The listing builds one solid part. Answer for the finished solid, in the listing's coordinates (mm). A direction names the side the tool comes from. Coordinates: 2 decimals unless noted, no trailing zeros. Order: outer loops, then holes, each group sorted by start corner. A loop starts at its lowest first (then second) coordinate and runs counter-clockwise, first axis right, second up. Notation, with made-up numbers: (23, 21.25) -> (73, 21.25) arc R28 cw to (73, 56.25) -> close; hole circle Ø2 at (-27, 36). An arc over 180 degrees is marked (long way). Write item = value, one per line. Start each with the question number.
```python
from build123d import *

# Parameters (mm, degrees)
SKETCH_1_R      = 32.5
EXTRUDE_1_DEPTH = 25
SKETCH_2_R      = 34.5
SKETCH_2_R_2    = 32.5
EXTRUDE_2_DEPTH = 20
FILLET_1_R      = 1
CHAMFER_1_SIZE  = 2


with BuildPart() as part:
    # 草图1 → 凸台-拉伸1 (new, symmetric)
    with BuildSketch(Plane(origin=(0, 0, 0), x_dir=(0, 0, -1), z_dir=(1, 0, 0))):
        Circle(SKETCH_1_R)
        with BuildLine():
            Line((5, 17.291616466), (5, 20.591616466))
            Line((5, 20.591616466), (-5, 20.591616466))
            Line((-5, 20.591616466), (-5, 17.291616466))
            ThreePointArc((-5, 17.291616466), (0, -18), (5, 17.291616466))
        make_face(mode=Mode.SUBTRACT)
    extrude(amount=EXTRUDE_1_DEPTH, both=True)

    # 草图2 → 凸台-拉伸2 (add, symmetric)
    with BuildSketch(Plane(origin=(0, 0, 0), x_dir=(0, 0, -1), z_dir=(1, 0, 0))):
        Circle(SKETCH_2_R)
        Circle(SKETCH_2_R_2, mode=Mode.SUBTRACT)
    extrude(amount=EXTRUDE_2_DEPTH, both=True)

    # 圆角1
    fillet_1_edges = [part.edges().sort_by_distance(p)[0] for p in [
        (-20, 0, 32.5),
        (20, 0, 32.5),
    ]]
    fillet(fillet_1_edges, radius=FILLET_1_R)

    # 倒角1
    chamfer_1_edges = [part.edges().sort_by_distance(p)[0] for p in [
        (-25, 0, 32.5),
        (25, 0, 32.5),
    ]]
    chamfer(chamfer_1_edges, length=CHAMFER_1_SIZE)


solid = part.part
```
Item 1: Each of these flat-tipped pins is pushed along its axis until it touches: pin 1 (1 mm diameter, centred on x = -17, z = 2, fed in from +Y); pin 2 (1 mm diameter, centred on x = -4.5, y = 8, fed in from +Z); pin 3 (6 mm diameter, centred on x = 6, z = 24.5, fed in from +Y); pin 4 (21.5 mm diameter, centred on y = 0, z = 0, fed in from +X). Where does it stop, or does it pass through?
Item 2: Section C-C, the plane x = 0 is taken. Give the vertices of the cut face in (y, z).
Item 3: Consider probe 1 along Y at (x, z) = (12, 0); probe 2 along Y at (x, z) = (-4, 9); probe 3 along Z at (x, y) = (12.5, -15.5). Determine where each line is inside the solid, lowest interval first.
Item 4: Section B-B, the plane z = 0 is taken. Give the vertices of the cut face in (x, y).
Item 5: Which of the six approach directions +Z, -Z, +X, -X, +Y, -Y give full straight-line access (tool end or side, diameter ignored) to faces 1 (the cylindrical face through (22.01, 9.76, -31)), 2 (the flat face through (0, 19, -5)), 3 (the flat face through (-20, 33.4, 5.3))?
Item 6: Section A-A, the plane y = 0 is taken. Give the vertices of the cut face in (x, z).
A:
q1.pin_1 = 34.47
q1.pin_2 = 33.67
q1.pin_3 = 26.98
q1.pin_4 = through
q2.outline = circle Ø69 at (0, 0); hole (17.29, -5) -> (20.59, -5) -> (20.59, 5) -> (17.29, 5) arc R18 ccw (long way) to start
q3.probe_1 = -34.5 to -18, 20.59 to 34.5
q3.probe_2 = -33.31 to -15.59, 15.59 to 33.31
q3.probe_3 = -30.82 to -9.15, 9.15 to 30.82
q4.outline = (-25, -30.5) -> (-23, -32.5) -> (-21, -32.5) arc R1 cw to (-20, -33.5) -> (-20, -34.5) -> (20, -34.5) -> (20, -33.5) arc R1 cw to (21, -32.5) -> (23, -32.5) -> (25, -30.5) -> (25, -18) -> (-25, -18) -> close; (-25, 20.59) -> (25, 20.59) -> (25, 30.5) -> (23, 32.5) -> (21, 32.5) arc R1 cw to (20, 33.5) -> (20, 34.5) -> (-20, 34.5) -> (-20, 33.5) arc R1 cw to (-21, 32.5) -> (-23, 32.5) -> (-25, 30.5) -> close
q5.face_1 = +X
q5.face_2 = +X, -X
q5.face_3 = -X
q6.outline = (-25, -30.5) -> (-23, -32.5) -> (-21, -32.5) arc R1 cw to (-20, -33.5) -> (-20, -34.5) -> (20, -34.5) -> (20, -33.5) arc R1 cw to (21, -32.5) -> (23, -32.5) -> (25, -30.5) -> (25, -18) -> (-25, -18) -> close; (-25, 18) -> (25, 18) -> (25, 30.5) -> (23, 32.5) -> (21, 32.5) arc R1 cw to (20, 33.5) -> (20, 34.5) -> (-20, 34.5) -> (-20, 33.5) arc R1 cw to (-21, 32.5) -> (-23, 32.5) -> (-25, 30.5) -> close
